Here's how the part is built. I have some questions about the finished solid (model axes, mm). A direction names the side the tool comes from. Round coordinates to 2 decimals unless told otherwise and drop trailing zeros. Order: outer loops, then holes, each group sorted by start corner. A loop starts at its lowest first (then second) coordinate and runs counter-clockwise, first axis right, second up. Notation, with made-up numbers: (19.5, 49) -> (29.5, 49) arc R21 cw to (29.5, 61) -> close; hole circle Ø11 at (-7.5, -13.75). An arc over 180 degrees is marked (long way). One line per item, written item: value.
```python
from build123d import *

# Parameters (mm, degrees)
FRONT_LUG_DEPTH            = 20
REAR_LUG_DEPTH             = 20
CONNECTING_BLOCK_PROFILE_W = 48
CONNECTING_BLOCK_PROFILE_H = 32
CONNECTING_BLOCK_DEPTH     = 12
CLEVIS_FORK_DEPTH          = 20
PIN_HOLE_PROFILE_R         = 11
PIN_HOLE_DEPTH             = 99


with BuildPart() as part:
    # Front Lug Profile → Front Lug (new body)
    with BuildSketch(Plane.XY):
        with BuildLine():
            Line((24, 0), (24, 36))
            Line((24, 36), (-24, 36))
            Line((-24, 36), (-24, 0))
            ThreePointArc((-24, 0), (0, -24), (24, 0))
        make_face()
    extrude(amount=-FRONT_LUG_DEPTH)



with BuildPart() as body_2:
    # Rear Lug Profile → Rear Lug (new body)
    with BuildSketch(Plane(origin=(0, 0, -52), x_dir=(-1, 0, 0), z_dir=(0, 0, -1))):
        with BuildLine():
            Line((-24, 0), (-24, 36))
            Line((-24, 36), (24, 36))
            Line((24, 36), (24, 0))
            ThreePointArc((24, 0), (0, -24), (-24, 0))
        make_face()
    extrude(amount=REAR_LUG_DEPTH)


with BuildPart() as part_1:
    add(part.part)

    add(body_2.part)  # Connecting Block merges body 2
    # Connecting Block Profile → Connecting Block (add)
    with BuildSketch(Plane(origin=(0, 36, 0), x_dir=(1, 0, 0), z_dir=(0, 1, 0))):
        with Locations((0, 36)):
            Rectangle(CONNECTING_BLOCK_PROFILE_W, CONNECTING_BLOCK_PROFILE_H)
    extrude(amount=-CONNECTING_BLOCK_DEPTH)

    # Clevis Fork Profile → Clevis Fork (add)
    with BuildSketch(Plane(origin=(0, 0, -72), x_dir=(-1, 0, 0), z_dir=(0, 0, -1))):
        with BuildLine():
            Line((10, 56), (10, 64))
            Line((10, 64), (24, 64))
            Line((24, 64), (24, 36))
            Line((24, 36), (-24, 36))
            Line((-24, 36), (-24, 64))
            Line((-24, 64), (-10, 64))
            Line((-10, 64), (-10, 56))
            ThreePointArc((-10, 56), (0, 46), (10, 56))
        make_face()
    extrude(amount=-CLEVIS_FORK_DEPTH)

    # Pin Hole Profile → Pin Hole (cut)
    with BuildSketch(Plane.XY):
        with Locations(Location((0, 0, 0), (0, 0, 180))):
            Circle(PIN_HOLE_PROFILE_R)
    extrude(amount=-PIN_HOLE_DEPTH, mode=Mode.SUBTRACT)


solid = part_1.part
```
Q1. For P1, Ø5, axis at x = -0.5, y = 11, coming from the +Z side; P2, Ø8.5, axis at x = 0, y = 47, coming from the +Z side; P3, Ø1.5, axis at x = 5, z = -25.5, coming from the -Y side; P4, Ø4, axis at y = -3, z = -60, coming from the -X side, each with a flat end and sliding along its axis, tell me the tip position at first contact or that it passes through.
Answers:
P1: z = 0
P2: z = -52
P3: y = 24
P4: x = -23.98
Q2. I need wall thicknesses on line 1 along Z through (x, y) = (-14, -13); line 2 along Y through (x, z) = (0, -55.75); line 3 along Y through (x, z) = (0, -19). Which ranges of each line are inside material? Lowest first, please.
Answers:
line 1: -72 to -52, -20 to 0
line 2: -24 to -11, 11 to 46
line 3: -24 to -11, 11 to 36
Q3. I want a section at B-B on z = -65. Write out the boundary of the cut face in (x, y).
Answers:
outline: (-24, 0) arc R24 ccw to (24, 0) -> (24, 64) -> (10, 64) -> (10, 56) arc R10 cw to (-10, 56) -> (-10, 64) -> (-24, 64) -> close; hole circle Ø22 at (0, 0)
Q4. I want a section at D-D on y = 53. Write out the boundary of the cut face in (x, z).
Answers:
outline: (-24, -72) -> (-9.54, -72) -> (-9.54, -52) -> (-24, -52) -> close; (9.54, -72) -> (24, -72) -> (24, -52) -> (9.54, -52) -> close
Q5. If we mould it in two halves opening along Y, with no side actions, what happens to faces 4 (the face through (17, 64, -62)), 5 (the face through (10, 60, -62)), 6 (the face through (2.38, 10.74, -9.86))? For each: pulls with the +Y half, pulls with the -Y half, needs draft (parallel to the pull), parting line crosses it, or undercut.
Answers:
face 4: pulls with the +Y half
face 5: needs draft
face 6: undercut
Q6. I want a section at A-A on x = 0. Write out the boundary of the cut face in (y, z), then the cut area to 3 significant figures.
Answers:
outline: (-24, -72) -> (-11, -72) -> (-11, -52) -> (-24, -52) -> close; (-24, -20) -> (-11, -20) -> (-11, 0) -> (-24, 0) -> close; (11, -72) -> (46, -72) -> (46, -52) -> (36, -52) -> (36, 0) -> (11, 0) -> (11, -20) -> (24, -20) -> (24, -52) -> (11, -52) -> close
area: 2,100 mm2
Q7. I want a section at C-C on y = -1. Write out the boundary of the cut face in (x, z).
Answers:
outline: (-23.98, -72) -> (-10.95, -72) -> (-10.95, -52) -> (-23.98, -52) -> close; (-23.98, -20) -> (-10.95, -20) -> (-10.95, 0) -> (-23.98, 0) -> close; (10.95, -72) -> (23.98, -72) -> (23.98, -52) -> (10.95, -52) -> close; (10.95, -20) -> (23.98, -20) -> (23.98, 0) -> (10.95, 0) -> close
Q8. Which directions (+Z, -Z, +X, -X, +Y, -Y) give clear straight access to the entire face, cutting with the end or side of a thin tool? Please do faces 1 (the face through (-10, 60, -62)), 2 (the face through (0, 44, -52)), 3 (the face through (5, 11, -52)).
Answers:
face 1: +Z, -Z, +Y
face 2: +Z, +X, -X, +Y
face 3: +X, -X, -Y
